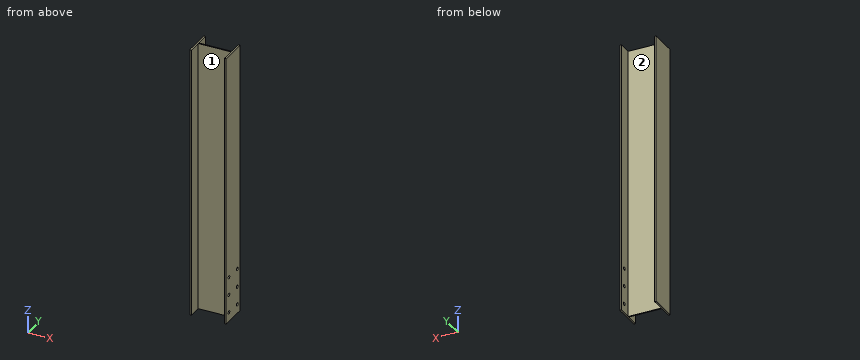
```python
from build123d import *

# Parameters (mm, degrees)
BOSS_EXTRUDE1_DEPTH = 1500
SKETCH2_R           = 9
CUT_EXTRUDE1_DEPTH  = 1500


with BuildPart() as part:
    # Sketch1 → Boss-Extrude1 (new body)
    with BuildSketch(Plane.XY):
        Polygon((-91, -75), (-100, -75), (-100, 75), (-91, 75), (-91, 3), (91, 3), (91, 75), (100, 75), (100, -75), (91, -75), (91, -3), (-91, -3), align=None)
    extrude(amount=BOSS_EXTRUDE1_DEPTH)

    # Sketch2 → Cut-Extrude1 (cut)
    with BuildSketch(Plane.ZY.offset(-91)):
        with Locations((50, -45)):
            Circle(SKETCH2_R)
        with Locations((150, -45)):
            Circle(SKETCH2_R)
        with Locations((250, -45)):
            Circle(SKETCH2_R)
        with Locations(Location((250, 45, 0), (0, 0, 270))):
            Circle(SKETCH2_R)
        with Locations(Location((150, 45, 0), (0, 0, 270))):
            Circle(SKETCH2_R)
        with Locations(Location((50, 45, 0), (0, 0, 270))):
            Circle(SKETCH2_R)
    extrude(amount=-CUT_EXTRUDE1_DEPTH, mode=Mode.SUBTRACT)


solid = part.part
```
Input: part model. Units: mm. Frame: model coordinates. Face numbers are marked on the shaded views. A direction names the side the tool comes from. Round coordinates to 2 decimals unless told otherwise and drop trailing zeros. Loops run counter-clockwise (first coordinate to the right, second up) from the corner with the lowest first, then second, coordinate; pieces in that order, holes last. Notation, with made-up numbers: (-12.75, 0.25) -> (-3.75, 0.25) arc R23 cw to (-3.75, 38.25) -> close; hole circle Ø6 at (79, 57.25). An arc over 180 degrees is marked (long way). Use one line per item in the form item = value. Start each with the question number.
Item 1: Section query C-C on x = -69.5. Return the cut outline in (y, z), then the cut area to 3 significant figures.
Item 2: Set-up query: the marked faces 1 and 2. Return all of +Z, -Z, +X, -X, +Y, -Y with unobstructed straight access to the full face (end or side cutting, diameter ignored); none if empty.
Item 3: Section query B-B on z = 94.5. Return the cut outline in (x, y).
Item 4: Section query A-A on y = -15.5. Return the cut outline in (x, z), then the cut area to 3 significant figures.
Item 5: Contact query for flat-ended pins moving along their axis: pin 1 Ø5 at (x, z) = (25, 690.5) entering from +Y; pin 2 Ø20.5 at (y, z) = (-45, 250) entering from +X; pin 3 Ø1 at (x, z) = (20.5, 827.5) entering from -Y. Output: stop coordinate, or through.
Item 6: Material intervals for L1, parallel to X at y = 14, z = 1332; L2, parallel to Y at x = -15, z = 1412, sorted ascending. Write a range as from..to.
Ans:
q1.outline = (-3, 0) -> (3, 0) -> (3, 1500) -> (-3, 1500) -> close
q1.area = 9,000 mm^2
q2.face_1 = +Z, -Z, -Y
q2.face_2 = +Z, -Z, +Y
q3.outline = (-100, -75) -> (-91, -75) -> (-91, -3) -> (91, -3) -> (91, -75) -> (100, -75) -> (100, 75) -> (91, 75) -> (91, 3) -> (-91, 3) -> (-91, 75) -> (-100, 75) -> close
q4.outline = (-100, 0) -> (-91, 0) -> (-91, 1500) -> (-100, 1500) -> close; (91, 0) -> (100, 0) -> (100, 1500) -> (91, 1500) -> close
q4.area = 27,000 mm^2
q5.pin_1 = 3
q5.pin_2 = 100
q5.pin_3 = -3
q6.L1 = -100..-91, 91..100
q6.L2 = -3..3
